Can you work these out from the model? Positions are in its coordinate system, mm. Give positions to 0.01 mm unless a question says otherwise; leave off trailing zeros. Order: outer loops, then holes, each group sorted by start corner. A loop starts at its lowest first (then second) coordinate and runs counter-clockwise, first axis right, second up.
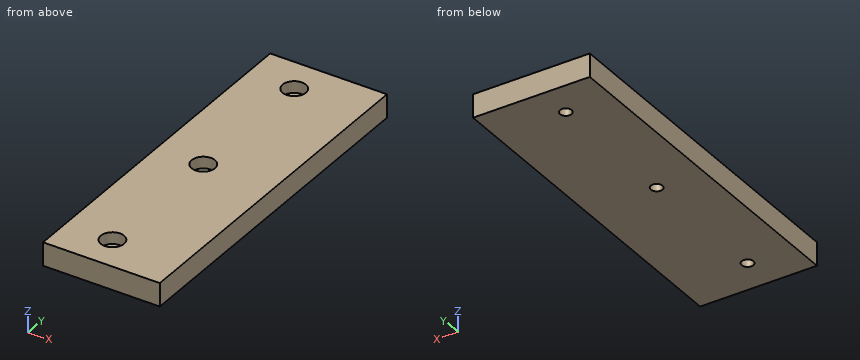
```python
from build123d import *

# Parameters (mm, degrees)
SKETCH1_W           = 50
SKETCH1_H           = 150
BOSS_EXTRUDE1_DEPTH = 5
HOLE1_D             = 5
HOLE1_CBORE_D       = 10
HOLE1_CBORE_DEPTH   = 5


with BuildPart() as part:
    # Sketch1 → Boss-Extrude1 (new, symmetric)
    with BuildSketch(Plane.XY):
        Rectangle(SKETCH1_W, SKETCH1_H)
    extrude(amount=BOSS_EXTRUDE1_DEPTH, both=True)

    # Hole1 (through all)
    with Locations(Plane.XY.offset(5)):
        with Locations((-5, 60), (-5, -60), (-5, 0)):
            CounterBoreHole(HOLE1_D / 2, HOLE1_CBORE_D / 2, HOLE1_CBORE_DEPTH)


solid = part.part
```
1) I'm going to push a flat-ended pin straight in: pin 1 Ø8 at (x, y) = (-5, 0) entering from +Z. Where does the tip first touch, or does it pass through?
2) Suppose I cut it at B-B (x = -5). Please give me the cut outline in (y, z).
3) Suppose I cut it at C-C (z = 1.5). Please give me the cut outline in (x, y).
4) If I drill on line 1 (Y direction, x = -5, z = 2.25); line 2 (Y direction, x = -1, z = 3.5); line 3 (X direction, y = 2.5, z = 2.5), over which ranges is the centre line in solid material (lowest first)?
5) Suppose I cut it at A-A (y = -60). Please give me the cut outline in (x, z).
Results:
1. pin 1: stops at z = 0
2. outline: (-75, -5) - (-62.5, -5) - (-62.5, 0) - (-65, 0) - (-65, 5) - (-75, 5) - close; (-57.5, -5) - (-2.5, -5) - (-2.5, 0) - (-5, 0) - (-5, 5) - (-55, 5) - (-55, 0) - (-57.5, 0) - close; (2.5, -5) - (57.5, -5) - (57.5, 0) - (55, 0) - (55, 5) - (5, 5) - (5, 0) - (2.5, 0) - close; (62.5, -5) - (75, -5) - (75, 5) - (65, 5) - (65, 0) - (62.5, 0) - close
3. outline: (-25, -75) - (25, -75) - (25, 75) - (-25, 75) - close; hole circle Ø10 at (-5, -60); hole circle Ø10 at (-5, 0); hole circle Ø10 at (-5, 60)
4. line 1: y = -75 to -65, -55 to -5, 5 to 55, 65 to 75
4. line 2: y = -75 to -63, -57 to -3, 3 to 57, 63 to 75
4. line 3: x = -25 to -9.33, -0.67 to 25
5. outline: (-25, -5) - (-7.5, -5) - (-7.5, 0) - (-10, 0) - (-10, 5) - (-25, 5) - close; (-2.5, -5) - (25, -5) - (25, 5) - (0, 5) - (0, 0) - (-2.5, 0) - close
